For this review, use the dimensioned drawing (mm, ordinates from the lowest corner) and the shaded views. Coordinates: 2 decimals unless noted, no trailing zeros. Loops run counter-clockwise (first coordinate to the right, second up) from the corner with the lowest first, then second, coordinate; pieces in that order, holes last. Notation, with made-up numbers: (57, 36.25) -> (62, 36.25) arc R30 cw to (62, 66.25) -> close; hole circle Ø10 at (80, 89.25). An arc over 180 degrees is marked (long way). Use one line per item in the form item = value. Start each with the question number.
1. Consider section D-D (x = 6.5). State the section outline as (y, z) points (1 decimal), then the cut area to 3 significant figures.
2. Consider section A-A (y = 4.75). State the section outline as (x, z) points.
3. The part is to be moulded in two halves that separate along Y. For the marked faces 1, 2, 3 and 4, say which applies: released by +Y, released by -Y, zero draft, split by the parting line, or undercut.
4. Consider section B-B (x = 9.5). State the section outline as (y, z) points (1 decimal).
5. Wall thickness on line 1 (Y direction, x = 10.25, z = 0.1) (1 decimal); line 2 (Y direction, x = 3.25, z = 0.6) (1 decimal); line 3 (Y direction, x = 6.5, z = 0.2) (1 decimal): over which ranges is each line inside the solid? List them lowest first. Write a range as from..to.
6. Consider section C-C (z = 0.25). State how many separate pieces and enclosed holes the cut face has.
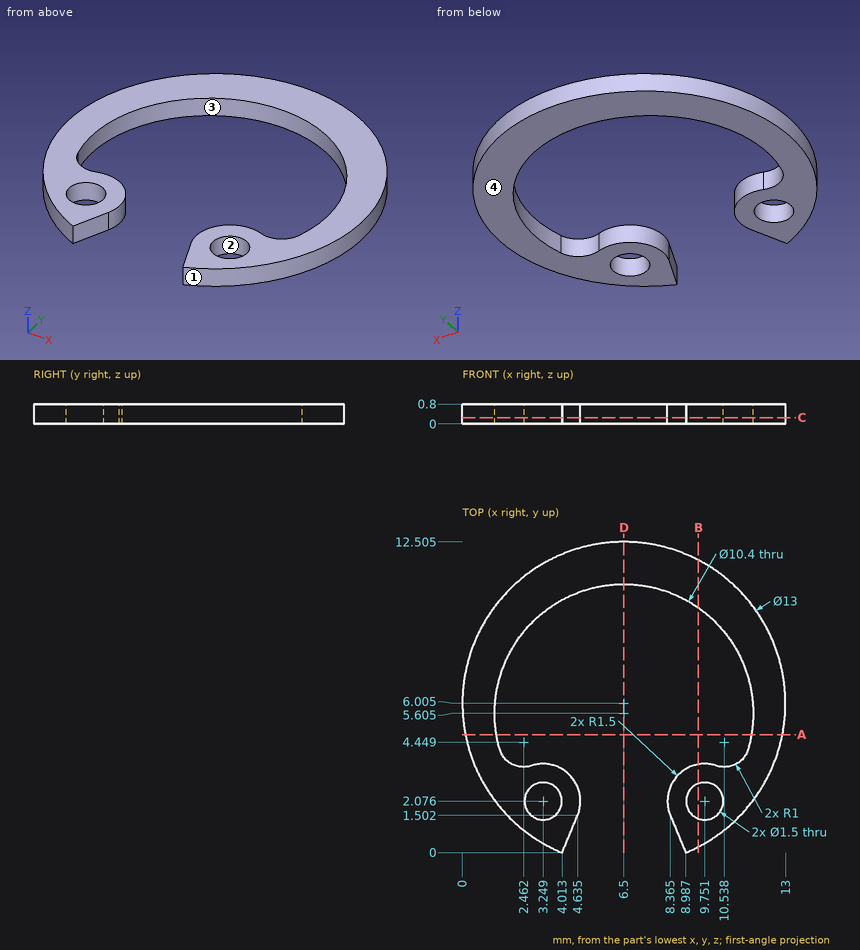
Geometry check:
q1.outline = (10.8, 0) -> (12.5, 0) -> (12.5, 0.8) -> (10.8, 0.8) -> close
q1.area = 1.36 mm²
q2.outline = (0.12, 0) -> (1.37, 0) -> (1.37, 0.8) -> (0.12, 0.8) -> close; (11.63, 0) -> (12.88, 0) -> (12.88, 0.8) -> (11.63, 0.8) -> close
q3.face_1 = split by the parting line
q3.face_2 = undercut
q3.face_3 = undercut
q3.face_4 = zero draft
q4.outline = (0.2, 0) -> (1.4, 0) -> (1.4, 0.8) -> (0.2, 0.8) -> close; (2.8, 0) -> (3.6, 0) -> (3.6, 0.8) -> (2.8, 0.8) -> close; (9.9, 0) -> (11.8, 0) -> (11.8, 0.8) -> (9.9, 0.8) -> close
q5.line_1 = 0.7..1.5, 2.6..3.5, 9.2..11.3
q5.line_2 = 0.4..1.3, 2.8..3.6, 9.7..11.6
q5.line_3 = 10.8..12.5
q6.separate_pieces = 1
q6.enclosed_holes = 2
